```python
from build123d import *

# Parameters (mm, degrees)
SKETCH1_R           = 1.6
SKETCH1_R_2         = 5.1
BOSS_EXTRUDE1_DEPTH = 6


with BuildPart() as part:
    # Sketch1 → Boss-Extrude1 (new body)
    with BuildSketch(Plane.XY):
        with BuildLine():
            Line((-45.309203126, -10.68796842), (-43.492395524, -11.905920573))
            ThreePointArc((-43.492395524, -11.905920573), (-42.764262434, -12.595973377), (-42.304336877, -13.487499682))
            ThreePointArc((-42.304336877, -13.487499682), (0.05, -44.45), (42.404336877, -13.487499682))
            ThreePointArc((42.404336877, -13.487499682), (42.864262434, -12.595973377), (43.592395524, -11.905920573))
            Line((43.592395524, -11.905920573), (45.409203126, -10.68796842))
            ThreePointArc((45.409203126, -10.68796842), (46.243586183, -9.847021456), (46.68737785, -8.748642725))
            ThreePointArc((46.68737785, -8.748642725), (47.5, 0), (46.68737785, 8.748642725))
            ThreePointArc((46.68737785, 8.748642725), (46.243586183, 9.847021456), (45.409203126, 10.68796842))
            Line((45.409203126, 10.68796842), (43.592395524, 11.905920573))
            ThreePointArc((43.592395524, 11.905920573), (42.864262434, 12.595973377), (42.404336877, 13.487499682))
            ThreePointArc((42.404336877, 13.487499682), (0.05, 44.45), (-42.304336877, 13.487499682))
            ThreePointArc((-42.304336877, 13.487499682), (-42.764262434, 12.595973377), (-43.492395524, 11.905920573))
            Line((-43.492395524, 11.905920573), (-45.309203126, 10.68796842))
            ThreePointArc((-45.309203126, 10.68796842), (-46.143586183, 9.847021456), (-46.58737785, 8.748642725))
            ThreePointArc((-46.58737785, 8.748642725), (-47.4, 0), (-46.58737785, -8.748642725))
            ThreePointArc((-46.58737785, -8.748642725), (-46.143586183, -9.847021456), (-45.309203126, -10.68796842))
        make_face()
        with Locations((-35.695198541, 20.6375)):
            Circle(SKETCH1_R, mode=Mode.SUBTRACT)
        with Locations((-35.695198541, -20.6375)):
            Circle(SKETCH1_R, mode=Mode.SUBTRACT)
        with Locations((35.795198541, -20.6375)):
            Circle(SKETCH1_R, mode=Mode.SUBTRACT)
        with Locations((35.795198541, 20.6375)):
            Circle(SKETCH1_R, mode=Mode.SUBTRACT)
        with Locations((12.777922061, 12.727922061)):
            Circle(SKETCH1_R_2, mode=Mode.SUBTRACT)
        with Locations((12.777922061, -12.727922061)):
            Circle(SKETCH1_R_2, mode=Mode.SUBTRACT)
        with Locations((-12.677922061, -12.727922061)):
            Circle(SKETCH1_R_2, mode=Mode.SUBTRACT)
        with Locations((-12.677922061, 12.727922061)):
            Circle(SKETCH1_R_2, mode=Mode.SUBTRACT)
        with Locations((0.05, -41.275)):
            Circle(SKETCH1_R, mode=Mode.SUBTRACT)
        with Locations((0.05, 41.275)):
            Circle(SKETCH1_R, mode=Mode.SUBTRACT)
    extrude(amount=BOSS_EXTRUDE1_DEPTH)


solid = part.part
```
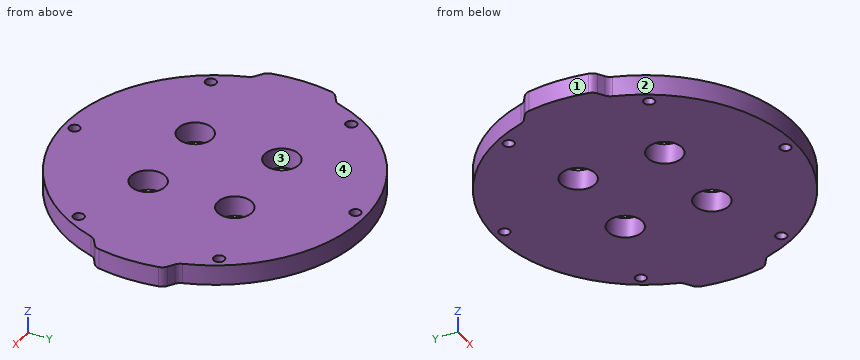
Design review of the part built by this model. Coordinates are the model's own, in mm. Face numbers are marked on the shaded views. Coordinates: 2 decimals unless noted, no trailing zeros. Order: outer loops, then holes, each group sorted by start corner. A loop starts at its lowest first (then second) coordinate and runs counter-clockwise, first axis right, second up. Notation, with made-up numbers: (-34.75, 81) -> (1.25, 81) arc R19 cw to (1.25, 101) -> close; hole circle Ø10 at (1, 3.5). An arc over 180 degrees is marked (long way). One line per item, written item: value. Start each with the question number.
Q1. Take a section at B-B, the plane z = 2. Give the number of separate pieces and of enclosed holes in the cut face, then the cut area to 3 significant figures.
Q2. For probe 1 along Y at (x, z) = (0.05, 2.3) (3 decimals); probe 2 along X at (y, z) = (12.5, 2.85); probe 3 along X at (y, z) = (-20, 3.4), list the stretches that pass through material, from the lowest coordinate up.
Q3. Insertion check: pin 1 Ø2 at (x, z) = (31.5, 3) entering from +Y; pin 2 Ø2 at (x, z) = (22, 3) entering from -Y; pin 3 Ø11.5 at (x, y) = (-12.68, -12.73) entering from +Z; pin 4 Ø1.5 at (x, z) = (17, 4) entering from +Y. Each pin has a flat end and moves straight along its axis. Give the tip position at first contact, or say it passes through.
Q4. Mouldability with a two-part tool opening along Y and no side actions: class the marked faces 1, 2, 3 and 4 as pulls with the +Y half, pulls with the -Y half, needs draft (parallel to the pull), parting line crosses it, or undercut.
Q5. Take a section at D-D, the plane y = 34. State the section outline as (x, z) points.
Q6. Take a section at A-A, the plane x = 13. State the section outline as (y, z) points, then the cut area to 3 significant figures.
Q7. Take a section at C-C, the plane x = 0.05. State the section outline as (y, z) points (3 decimals).
Values follow:
1. separate pieces: 1
1. enclosed holes: 10
1. area: 5,970 mm2
2. probe 1: y = -44.45 to -42.875, -39.675 to 39.675, 42.875 to 44.45
2. probe 2: x = -42.84 to -17.77, -7.58 to 7.68, 17.87 to 42.94
2. probe 3: x = -39.65 to -37.16, -34.23 to 34.33, 37.26 to 39.75
3. pin 1: stops at y = 32.38
3. pin 2: stops at y = -39.2
3. pin 3: stops at z = 6
3. pin 4: stops at y = 41.39
4. face 1: parting line crosses it
4. face 2: pulls with the -Y half
4. face 3: undercut
4. face 4: needs draft
5. outline: (-28.58, 0) -> (28.68, 0) -> (28.68, 6) -> (-28.58, 6) -> close
6. outline: (-42.52, 0) -> (-17.82, 0) -> (-17.82, 6) -> (-42.52, 6) -> close; (-7.63, 0) -> (7.63, 0) -> (7.63, 6) -> (-7.63, 6) -> close; (17.82, 0) -> (42.52, 0) -> (42.52, 6) -> (17.82, 6) -> close
6. area: 388 mm2
7. outline: (-44.45, 0) -> (-42.875, 0) -> (-42.875, 6) -> (-44.45, 6) -> close; (-39.675, 0) -> (39.675, 0) -> (39.675, 6) -> (-39.675, 6) -> close; (42.875, 0) -> (44.45, 0) -> (44.45, 6) -> (42.875, 6) -> close
